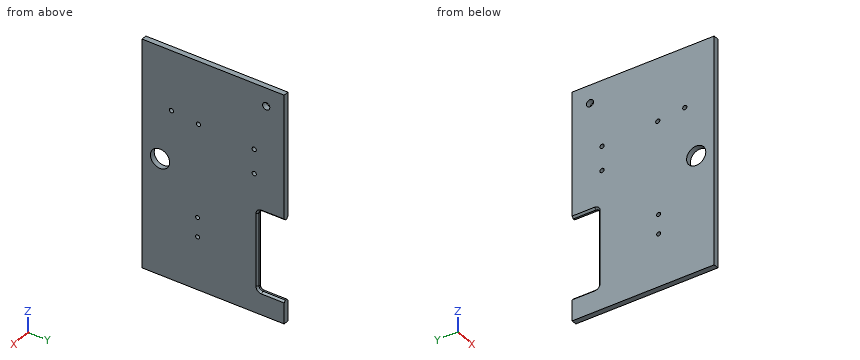
```python
from build123d import *

# Parameters (mm, degrees)
BOSS_EXTRUDE1_DEPTH = 22.5
SKETCH2_R           = 30
SKETCH2_R_2         = 17.5
SKETCH2_R_3         = 80
CUT_EXTRUDE1_DEPTH  = 1812.9464672
FILLET1_R           = 31
CHAMFER1_SIZE       = 15
SKETCH3_R           = 16.5
CUT_EXTRUDE2_DEPTH  = 159


with BuildPart() as part:
    # Sketch1 → Boss-Extrude1 (new, symmetric)
    with BuildSketch(Plane(origin=(0, 0, 0), x_dir=(0, 0, -1), z_dir=(1, 0, 0))):
        Polygon((0, 0), (520, 0), (520, 1185), (331, 1185), (331, 965), (-331, 965), (-331, 1185), (-1370, 1185), (-1370, 0), align=None)
    extrude(amount=BOSS_EXTRUDE1_DEPTH, both=True)

    # Sketch2 → Cut-Extrude1 (cut, through all)
    with BuildSketch(Plane(origin=(22.5, 0, 0), x_dir=(0, 0, -1), z_dir=(1, 0, 0))):
        with Locations((-1220, 1035)):
            Circle(SKETCH2_R)
        with Locations((-825, 935)):
            Circle(SKETCH2_R_2)
        with Locations((-625, 935)):
            Circle(SKETCH2_R_2)
        with Locations((-850, 470)):
            Circle(SKETCH2_R_2)
        with Locations((-875, 245)):
            Circle(SKETCH2_R_2)
        with Locations((-440, 150)):
            Circle(SKETCH2_R_3)
    extrude(amount=-CUT_EXTRUDE1_DEPTH, mode=Mode.SUBTRACT)

    # Fillet1
    fillet1_edges = [part.edges().sort_by_distance(p)[0] for p in [
        (0, 965, 331),
        (0, 965, -331),
    ]]
    fillet(fillet1_edges, radius=FILLET1_R)

    # Chamfer1
    chamfer1_edges = [part.edges().sort_by_distance(p)[0] for p in [
        (-22.5, 1090.5, -331),
        (22.5, 1090.5, -331),
        (-22.5, 965, 0),
        (22.5, 965, 0),
        (-22.5, 1090.5, 331),
        (22.5, 1090.5, 331),
        (-22.5, 974.079689783, -321.920310217),
        (22.5, 974.079689783, -321.920310217),
        (-22.5, 974.079689783, 321.920310217),
        (22.5, 974.079689783, 321.920310217),
    ]]
    chamfer(chamfer1_edges, length=CHAMFER1_SIZE)

    # Sketch3 → Cut-Extrude2 (cut)
    with BuildSketch(Plane(origin=(22.5, 0, 0), x_dir=(0, 0, -1), z_dir=(1, 0, 0))):
        with Locations((-77, 463)):
            Circle(SKETCH3_R)
        with Locations((83, 463)):
            Circle(SKETCH3_R)
    extrude(amount=-CUT_EXTRUDE2_DEPTH, mode=Mode.SUBTRACT)


solid = part.part
```
For this review, take the finished solid that the model builds, in its own axes (mm). Coordinates: 2 decimals unless noted, no trailing zeros. Loops run counter-clockwise (first coordinate to the right, second up) from the corner with the lowest first, then second, coordinate; pieces in that order, holes last. Notation, with made-up numbers: (74, 64.5) - (126, 64.5) arc R33 cw to (126, 92.5) - close; hole circle Ø4 at (27, 56). An arc over 180 degrees is marked (long way). Use one line per item in the form item = value. Start each with the question number.
1) Take a section at A-A (y = 1035). State the section outline as (x, z) points, plus the area to 3 significant figures.
2) For pin 1 (7.5 mm diameter, centred on x = -3, z = 9.5, fed in from +Y), flat-tipped, find the tip position at first contact; note if it passes through.
3) Take a section at B-B (y = 150). State the section outline as (x, z) points.
4) To check wall thickness, follow probe 1 along Y at (x, z) = (9, 625.5); probe 2 along Y at (x, z) = (-12, 440); probe 3 along Z at (x, y) = (9, 1091.5). State the ranges of each line that lie inside material, in increasing order. Write a range as from..to.
5) Take a section at C-C (z = 444). State the section outline as (x, y) points.
From the geometry:
q1.outline = (-22.5, -520) - (22.5, -520) - (22.5, -346) - (7.5, -331) - (-7.5, -331) - (-22.5, -346) - close; (-22.5, 346) - (-7.5, 331) - (7.5, 331) - (22.5, 346) - (22.5, 1190) - (-22.5, 1190) - close; (-22.5, 1250) - (22.5, 1250) - (22.5, 1370) - (-22.5, 1370) - close
q1.area = 52,100 mm2
q2.pin_1 = 965
q3.outline = (-22.5, -520) - (22.5, -520) - (22.5, 360) - (-22.5, 360) - close; (-22.5, 520) - (22.5, 520) - (22.5, 1370) - (-22.5, 1370) - close
q4.probe_1 = 0..917.51, 952.49..1185
q4.probe_2 = 0..70, 230..1185
q4.probe_3 = -520..-332.5, 332.5..1370
q5.outline = (-22.5, 0) - (22.5, 0) - (22.5, 70.1) - (-22.5, 70.1) - close; (-22.5, 229.9) - (22.5, 229.9) - (22.5, 1185) - (-22.5, 1185) - close
